Part model, mm, in its own coordinate system. A direction names the side the tool comes from. Coordinates: 2 decimals unless noted, no trailing zeros. Loops run counter-clockwise (first coordinate to the right, second up) from the corner with the lowest first, then second, coordinate; pieces in that order, holes last. Notation, with made-up numbers: M 35.25,22.25 L 39.25,22.25 A30 cw 39.25,47.25 Z; hole C 65.5,72.5 d10. An arc over 180 degrees is marked long. Use a Markdown table: item, result. Add a question column.
1) Pin check, flat tip, straight feed: pin 1 Ø6 at (x, z) = (-26.5, -17.5) entering from -Y. Stop position of the tip, or through.
2) Wall check: probe 1 along Z at (x, y) = (26.5, 271); probe 2 along X at (y, z) = (1225, 7.5). Give the ranges that are in metal, low to high. Write a range as from..to.
3) Band-saw the part on B-B (z = 8). List the corners of the cut face in (x, y).
4) Band-saw the part on A-A (y = 184). List the corners of the cut face in (x, z), plus the area to 3 significant figures.
5) Pull direction Z, two halves, no side cores. Call faces 1 (the flat face through (30, 643, 0)), 2 (the flat face through (-0.49, 42.284, 30.621)), 3 (the flat face through (0, 644, -35)), 4 (the flat face through (-30, 654, 0)): released by +Z, released by -Z, zero draft, split by the parting line, or undercut.
6) Band-saw the part on C-C (x = -5). List the corners of the cut face in (y, z), plus the area to 3 significant figures.
7) Tool access for faces 5 (the flat face through (0, 644, -30)), 6 (the flat face through (-35, 655, 0)): list every direction of +Z, -Z, +X, -X, +Y, -Y with a clear straight run to the whole face (end or side of a thin tool).
from build123d import *

# Parameters (mm, degrees)
FEATURE_19_WELDMEMBERFEAT_4_MORE_IN_5_DEPTH = 1302
CUT_EXTRUDE1_DEPTH                          = 1305.350029708
CUT_EXTRUDE1_DEPTH_BACK                     = 1305.350029708


with BuildPart() as part:
    # Sketch1 → feature 19 (WeldMemberFeat) (+4 more in 5 files) Cold-formed Hollow Structural Square Steel(gb t6728-2002) 70×70×5(1) (new body)
    with BuildSketch(Plane(origin=(0, 0, 0), x_dir=(-1, 0, 0), z_dir=(0, 1, 0))):
        with BuildLine():
            Line((-25, -35), (25, -35))
            ThreePointArc((25, -35), (32.071067812, -32.071067812), (35, -25))
            Line((35, -25), (35, 25))
            ThreePointArc((35, 25), (32.071067812, 32.071067812), (25, 35))
            Line((25, 35), (-25, 35))
            ThreePointArc((-25, 35), (-32.071067812, 32.071067812), (-35, 25))
            Line((-35, 25), (-35, -25))
            ThreePointArc((-35, -25), (-32.071067812, -32.071067812), (-25, -35))
        make_face()
        with BuildLine():
            Line((-25, -30), (25, -30))
            ThreePointArc((25, -30), (28.535533906, -28.535533906), (30, -25))
            Line((30, -25), (30, 25))
            ThreePointArc((30, 25), (28.535533906, 28.535533906), (25, 30))
            Line((25, 30), (-25, 30))
            ThreePointArc((-25, 30), (-28.535533906, 28.535533906), (-30, 25))
            Line((-30, 25), (-30, -25))
            ThreePointArc((-30, -25), (-28.535533906, -28.535533906), (-25, -30))
        make_face(mode=Mode.SUBTRACT)
    extrude(amount=FEATURE_19_WELDMEMBERFEAT_4_MORE_IN_5_DEPTH)

    # 0:feat:20/0 feature 20/0 (ProfileFeature) (+11 more in 7 files) Sketch2 → Cut-Extrude1 (cut, two sides: drawn at the far end of the back side and taken through both)
    with BuildSketch(Plane.XY.offset(35).offset(-CUT_EXTRUDE1_DEPTH_BACK)):
        Polygon((35, 1302), (-35, 1243.247002398), (-35, 1302), align=None)
        Polygon((-35, 83.4), (35, 0), (-35, 0), align=None)
    extrude(amount=CUT_EXTRUDE1_DEPTH + CUT_EXTRUDE1_DEPTH_BACK, mode=Mode.SUBTRACT)


solid = part.part
Entries:
| question | item | result |
|---|---|---|
| 1 | pin 1 | through |
| 2 | probe 1 | -34.89..-29.77, 29.77..34.89 |
| 2 | probe 2 | -35..-30, 30..35 |
| 3 | outline | M -35,83.4 L -30,77.44 L -30,1247.44 L -35,1243.25 Z; M 30,5.96 L 35,0 L 35,1302 L 30,1297.8 Z |
| 4 | outline | M -35,-25 A10 ccw -25,-35 L 25,-35 A10 ccw 35,-25 L 35,25 A10 ccw 25,35 L -25,35 A10 ccw -35,25 Z; hole M -30,-25 A5 ccw -25,-30 L 25,-30 A5 ccw 30,-25 L 30,25 A5 ccw 25,30 L -25,30 A5 ccw -30,25 Z |
| 4 | area | 1,240 mm2 |
| 5 | face 1 | undercut |
| 5 | face 2 | zero draft |
| 5 | face 3 | released by -Z |
| 5 | face 4 | undercut |
| 6 | outline | M 47.66,-35 L 1268.43,-35 L 1268.43,-30 L 47.66,-30 Z; M 47.66,30 L 1268.43,30 L 1268.43,35 L 47.66,35 Z |
| 6 | area | 12,200 mm2 |
| 7 | face 5 | +Y, -Y |
| 7 | face 6 | +Z, -Z, -X, +Y, -Y |
